from build123d import *

# Parameters (mm, degrees)
SKETCH1_W                                           = 50
SKETCH1_H                                           = 12
BOSS_EXTRUDE1_DEPTH                                 = 7
HOLE_SIZE_PER_SOCKET_HEAD_CAP_SCREW_TYP_D           = 5.5
HOLE_SIZE_PER_SOCKET_HEAD_CAP_SCREW_TYP_CBORE_D     = 10
HOLE_SIZE_PER_SOCKET_HEAD_CAP_SCREW_TYP_CBORE_DEPTH = 5.7


with BuildPart() as part:
    # Sketch1 → Boss-Extrude1 (new, symmetric)
    with BuildSketch(Plane(origin=(0, 0, 0), x_dir=(1, 0, 0), z_dir=(0, 1, 0))):
        Rectangle(SKETCH1_W, SKETCH1_H)
    extrude(amount=BOSS_EXTRUDE1_DEPTH, both=True)

    # Hole Size (per socket head cap screw type)1 (through all)
    with Locations(Plane(origin=(0, 7, 0), x_dir=(1, 0, 0), z_dir=(0, 1, 0))):
        with Locations((15, 0), (-15, 0)):
            CounterBoreHole(HOLE_SIZE_PER_SOCKET_HEAD_CAP_SCREW_TYP_D / 2, HOLE_SIZE_PER_SOCKET_HEAD_CAP_SCREW_TYP_CBORE_D / 2, HOLE_SIZE_PER_SOCKET_HEAD_CAP_SCREW_TYP_CBORE_DEPTH)


solid = part.part
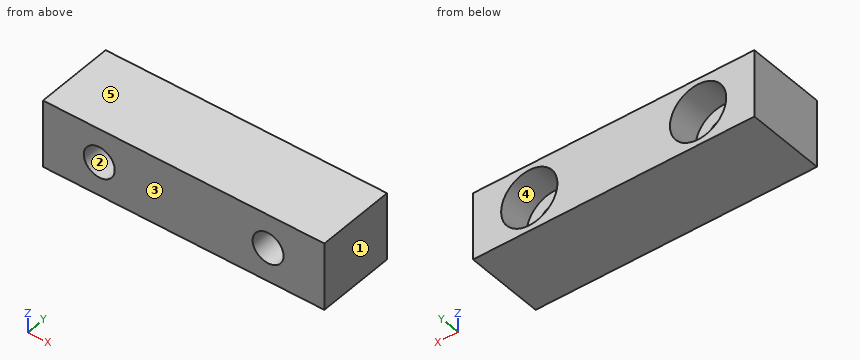
For this review, take the finished solid that the model builds, in its own axes (mm). Face numbers are marked on the shaded views. A direction names the side the tool comes from. Give positions to 0.01 mm unless a question says otherwise; leave off trailing zeros. Loops run counter-clockwise (first coordinate to the right, second up) from the corner with the lowest first, then second, coordinate; pieces in that order, holes last.
Item 1: Draft analysis for pull direction X (two halves, no side actions). For the marked faces 1, 2 and 3, state which applies: +X half, -X half, draft (parallel to the pull), parting line (faces both ways), or undercut.
Item 2: Take a section at D-D, the plane z = -4.5. State the section outline as (x, y) points, and give its area (3 significant figures).
Item 3: Take a section at B-B, the plane z = 0. State the section outline as (x, y) points.
Item 4: Take a section at C-C, the plane y = 2.5. State the section outline as (x, z) points.
Item 5: For line 1 along Z through (x, y) = (15, -3.25); line 2 along Z through (x, y) = (15, 5.6); line 3 along X through (y, z) = (5.75, -2.75), list the stretches that pass through material, from the lowest coordinate up.
Item 6: Insertion check: pin 1 (5 mm diameter, centred on x = -14.5, z = 0, fed in from +Y). The pin has a flat end and moves straight along its axis. Give the tip position at first contact, or say it passes through.
Item 7: Take a section at A-A, the plane x = 15. State the section outline as (y, z) points.
Item 8: Tool access review of the marked faces 4 and 5: name each direction out of +Z, -Z, +X, -X, +Y, -Y from which nothing blocks a thin tool from reaching the whole face with its end or side.
Calculated:
1. face 1: +X half
1. face 2: undercut
1. face 3: draft
2. outline: (-25, -7) - (25, -7) - (25, 7) - (17.18, 7) - (17.18, 1.3) - (12.82, 1.3) - (12.82, 7) - (-12.82, 7) - (-12.82, 1.3) - (-17.18, 1.3) - (-17.18, 7) - (-25, 7) - close
2. area: 650 mm2
3. outline: (-25, -7) - (-17.75, -7) - (-17.75, 1.3) - (-20, 1.3) - (-20, 7) - (-25, 7) - close; (-12.25, -7) - (12.25, -7) - (12.25, 1.3) - (10, 1.3) - (10, 7) - (-10, 7) - (-10, 1.3) - (-12.25, 1.3) - close; (17.75, -7) - (25, -7) - (25, 7) - (20, 7) - (20, 1.3) - (17.75, 1.3) - close
4. outline: (-25, -6) - (25, -6) - (25, 6) - (-25, 6) - close; hole circle Ø10 at (-15, 0); hole circle Ø10 at (15, 0)
5. line 1: z = -6 to -2.75, 2.75 to 6
5. line 2: z = -6 to -5, 5 to 6
5. line 3: x = -25 to -19.18, -10.82 to 10.82, 19.18 to 25
6. pin 1: stops at y = 1.3
7. outline: (-7, -6) - (7, -6) - (7, -5) - (1.3, -5) - (1.3, -2.75) - (-7, -2.75) - close; (-7, 2.75) - (1.3, 2.75) - (1.3, 5) - (7, 5) - (7, 6) - (-7, 6) - close
8. face 4: +Y
8. face 5: +Z, +X, -X, +Y, -Y
